from build123d import *

# Parameters (mm, degrees)
SKETCH1_W               = 5
SKETCH1_H               = 5
BOSS_EXTRUDE1_DEPTH     = 160
SKETCH2_W               = 10
SKETCH2_H               = 5
BOSS_EXTRUDE2_DEPTH     = 18
SKETCH3_W               = 5
SKETCH3_H               = 19.358131828
CUT_EXTRUDE1_DEPTH      = 12
CUT_EXTRUDE2_DEPTH      = 179.298205263
CUT_EXTRUDE2_DEPTH_BACK = 179.298205263
SKETCH4_R               = 1
SKETCH5_W               = 5
SKETCH5_H               = 5
BOSS_EXTRUDE3_DEPTH     = 190


with BuildPart() as part:
    # Sketch1 → Boss-Extrude1 (new body)
    with BuildSketch(Plane.XY):
        Rectangle(SKETCH1_W, SKETCH1_H)
    extrude(amount=BOSS_EXTRUDE1_DEPTH)

    # Sketch2 → Boss-Extrude2 (add)
    with BuildSketch(Plane.XY.offset(160)):
        Rectangle(SKETCH2_W, SKETCH2_H)
    extrude(amount=BOSS_EXTRUDE2_DEPTH)

    # Sketch3 → Cut-Extrude1 (cut)
    with BuildSketch(Plane.XY.offset(178)):
        Rectangle(SKETCH3_W, SKETCH3_H)
    extrude(amount=-CUT_EXTRUDE1_DEPTH, mode=Mode.SUBTRACT)

    # Sketch4 → Cut-Extrude2 (cut, two sides: drawn at the far end of the back side and taken through both)
    with BuildSketch(Plane(origin=(5, 0, 0), x_dir=(0, 0, -1), z_dir=(1, 0, 0)).offset(-CUT_EXTRUDE2_DEPTH_BACK)):
        with Locations(Location((-170, 0, 0), (0, 0, 90))):
            Circle(SKETCH4_R)
        with BuildLine():
            Line((-170, 2.5), (-170, 12.575428257))
            Line((-170, 12.575428257), (-197.273990227, 12.575428257))
            Line((-197.273990227, 12.575428257), (-202.218051786, -13.998902623))
            Line((-202.218051786, -13.998902623), (-170, -2.5))
            ThreePointArc((-170, -2.5), (-172.5, 0), (-170, 2.5))
        make_face()
    extrude(amount=CUT_EXTRUDE2_DEPTH + CUT_EXTRUDE2_DEPTH_BACK, mode=Mode.SUBTRACT)

    # Sketch5 → Boss-Extrude3 (add)
    with BuildSketch(Plane(origin=(0, 0, 0), x_dir=(1, 0, 0), z_dir=(0, 1, 0))):
        with Locations((0, -70)):
            Rectangle(SKETCH5_W, SKETCH5_H)
    extrude(amount=BOSS_EXTRUDE3_DEPTH)


solid = part.part
Build history of the part. All positions in model axes, mm. A direction names the side the tool comes from. Round coordinates to 2 decimals unless told otherwise and drop trailing zeros. Loops run counter-clockwise (first coordinate to the right, second up) from the corner with the lowest first, then second, coordinate; pieces in that order, holes last. Notation, with made-up numbers: (-30.5, 35) -> (-23.5, 35) arc R26 cw to (-23.5, 50) -> close; hole circle Ø1 at (18.25, 45). An arc over 180 degrees is marked (long way). One line per item, written item: value. Start each with the question number.
Q1. Drop flat-ended pins along their axis: pin 1 Ø2 at (x, y) = (-4, 1) entering from -Z; pin 2 Ø4 at (x, z) = (0, 21.5) entering from +Y; pin 3 Ø1.5 at (x, y) = (-0.5, 80) entering from -Z. Give the stop position or say it passes through.
Q2. Probe line 1 along Z through (x, y) = (3.1, 0); line 2 along Y through (x, z) = (-3.85, 170); line 3 along Y through (x, z) = (-2, 105). List the from-to ranges inside material, lowest first.
Q3. Two-plate mould, pull along X, no slides. Class faces 1 (the face through (2.5, 51, 69)), 2 (the face through (0, -2.5, 84)), 3 (the face through (0, 0, 166)): released by +X, released by -X, zero draft, split by the parting line, or undercut.
Q4. 3-axis set-ups, long thin cutter, end or side, ignore diameter. For faces 4 (the face through (-2.5, 51, 68)), 5 (the face through (2.5, 0, 168.6)), 6 (the face through (0, 2.5, 33)): which of +Z, -Z, +X, -X, +Y, -Y reach the whole face in a straight line?
Q5. Cut at A-A on x = 0. List the corners of the cut face in (y, z).
Q6. Cut at C-C on y = 147.5. List the corners of the cut face in (x, z), plus the area to 3 significant figures.
Q7. Cut at B-B on z = 80.5. List the corners of the cut face in (x, y).
Computed:
1. pin 1: z = 160
1. pin 2: y = 2.5
1. pin 3: z = 67.5
2. line 1: 160 to 169, 171 to 172.5
2. line 2: -2.5 to -1, 1 to 2.5
2. line 3: -2.5 to 2.5
3. face 1: released by +X
3. face 2: zero draft
3. face 3: undercut
4. face 4: -Z, -X, +Y, -Y
4. face 5: +Z, +Y, -Y
4. face 6: -Z, +X, -X, +Y
5. outline: (-2.5, 0) -> (2.5, 0) -> (2.5, 67.5) -> (190, 67.5) -> (190, 72.5) -> (2.5, 72.5) -> (2.5, 166) -> (-2.5, 166) -> close
6. outline: (-2.5, 67.5) -> (2.5, 67.5) -> (2.5, 72.5) -> (-2.5, 72.5) -> close
6. area: 25.0 mm²
7. outline: (-2.5, -2.5) -> (2.5, -2.5) -> (2.5, 2.5) -> (-2.5, 2.5) -> close
